```python
from build123d import *

# Parameters (mm, degrees)
SKETCH1_R           = 12.5
BOSS_EXTRUDE1_DEPTH = 58
SKETCH2_R           = 3
BOSS_EXTRUDE2_DEPTH = 3
SKETCH3_R           = 2
BOSS_EXTRUDE3_DEPTH = 9
SKETCH4_R           = 1.5
CUT_EXTRUDE1_DEPTH  = 6
CHAMFER1_SIZE       = 1
CHAMFER2_SIZE       = 1


with BuildPart() as part:
    # Sketch1 → Boss-Extrude1 (new body)
    with BuildSketch(Plane(origin=(0, 0, 0), x_dir=(0, 0, -1), z_dir=(1, 0, 0))):
        with Locations(Location((0, 0, 0), (0, 0, 180))):
            Circle(SKETCH1_R)
    extrude(amount=BOSS_EXTRUDE1_DEPTH)

    # Sketch2 → Boss-Extrude2 (add)
    with BuildSketch(Plane(origin=(58, 0, 0), x_dir=(0, 0, -1), z_dir=(1, 0, 0))):
        Circle(SKETCH2_R)
    extrude(amount=BOSS_EXTRUDE2_DEPTH)

    # Sketch3 → Boss-Extrude3 (add)
    with BuildSketch(Plane(origin=(61, 0, 0), x_dir=(0, 0, -1), z_dir=(1, 0, 0))):
        Circle(SKETCH3_R)
    extrude(amount=BOSS_EXTRUDE3_DEPTH)

    # Sketch4 → Cut-Extrude1 (cut)
    with BuildSketch(Plane(origin=(58, 0, 0), x_dir=(0, 0, -1), z_dir=(1, 0, 0))):
        with Locations((0, 8.5)):
            Circle(SKETCH4_R)
        with Locations(Location((0, -8.5, 0), (0, 0, 180))):
            Circle(SKETCH4_R)
    extrude(amount=-CUT_EXTRUDE1_DEPTH, mode=Mode.SUBTRACT)

    # Chamfer1
    chamfer1_edges = [part.edges().sort_by_distance(p)[0] for p in [
        (58, 0, -12.5),
    ]]
    chamfer(chamfer1_edges, length=CHAMFER1_SIZE)

    # Chamfer2
    chamfer2_edges = [part.edges().sort_by_distance(p)[0] for p in [
        (0, 0, -12.5),
    ]]
    chamfer(chamfer2_edges, length=CHAMFER2_SIZE)


solid = part.part
```
Check sheet for the modelled part. Datum: model origin and axes. Units: mm. A direction names the side the tool comes from. Round coordinates to 2 decimals unless told otherwise and drop trailing zeros. Loops run counter-clockwise (first coordinate to the right, second up) from the corner with the lowest first, then second, coordinate; pieces in that order, holes last. Notation, with made-up numbers: (-35.5, 60) - (-23.5, 60) arc R31 cw to (-23.5, 92) - close; hole circle Ø7 at (-29.75, 11). An arc over 180 degrees is marked (long way). Write item = value, one per line. Start each with the question number.
Q1. Section check B-B (y = 0). Record the boundary of the cut face in (x, z), plus the area to 3 significant figures.
Q2. Access from +Z, -Z, +X, -X, +Y, -Y to the whole of each face (thin tool, end or side, straight path). Record for faces 1 (the face through (59, 0, 3)), 2 (the face through (70, 0, 0)).
Q3. Depth check by flat-ended pin: P1, Ø4, axis at x = 19, z = -4.5, coming from the -Y side; P2, Ø8, axis at x = 53.5, y = 5, coming from the +Z side; P3, Ø1.5, axis at y = -8, z = 0, coming from the +X side. Enter the tip coordinate at first touch or a pass-through.
Q4. Thickness scan on L1, parallel to Y at x = 54.85, z = 0; L2, parallel to X at y = 10, z = 4.75; L3, parallel to Z at x = 56, y = -8. Record the ranges inside material, lowest first.
Q5. Release check for a two-part mould opening along Y. For faces 3 (the face through (61, -2, -1)), 4 (the face through (65, -2, 0)), 5 (the face through (52, -9, 0)) record: pulls with the +Y half, pulls with the -Y half, needs draft (parallel to the pull), parting line crosses it, or undercut.
Q6. Section check A-A (z = 0). Record the boundary of the cut face in (x, y), plus the area to 3 significant figures.
Q7. Section check C-C (x = 6). Record the boundary of the cut face in (y, z), plus the area to 3 significant figures.
Derived:
q1.outline = (0, -11.5) - (1, -12.5) - (57, -12.5) - (58, -11.5) - (58, -3) - (61, -3) - (61, -2) - (70, -2) - (70, 2) - (61, 2) - (61, 3) - (58, 3) - (58, 11.5) - (57, 12.5) - (1, 12.5) - (0, 11.5) - close
q1.area = 1,500 mm^2
q2.face_1 = +X
q2.face_2 = +Z, -Z, +X, +Y, -Y
q3.P1 = -12.25
q3.P2 = 12.46
q3.P3 = 52
q4.L1 = -12.5 to -10, -7 to 7, 10 to 12.5
q4.L2 = 0 to 58
q4.L3 = -9.6 to -1.41, 1.41 to 9.6
q5.face_3 = needs draft
q5.face_4 = parting line crosses it
q5.face_5 = undercut
q6.outline = (0, -11.5) - (1, -12.5) - (57, -12.5) - (58, -11.5) - (58, -10) - (52, -10) - (52, -7) - (58, -7) - (58, -3) - (61, -3) - (61, -2) - (70, -2) - (70, 2) - (61, 2) - (61, 3) - (58, 3) - (58, 7) - (52, 7) - (52, 10) - (58, 10) - (58, 11.5) - (57, 12.5) - (1, 12.5) - (0, 11.5) - close
q6.area = 1,470 mm^2
q7.outline = circle Ø25 at (0, 0)
q7.area = 491 mm^2
